Read the model definition and answer for the solid it produces. Units are mm, in the model's axes. Face numbers are marked on the shaded views. A direction names the side the tool comes from. Give positions to 0.01 mm unless a question says otherwise; leave off trailing zeros. Write each loop counter-clockwise with the first axis right and the second up, starting at its lowest first coordinate (ties: lowest second). Pieces come first, ordered by that corner, then holes. Notation, with made-up numbers: (33.25, -24.75) -> (74.25, -24.75) arc R22 ccw to (74.25, -16.75) -> close; hole circle Ø1 at (62, 11). An arc over 180 degrees is marked (long way). Answer as CSV lines item,"result". Start each with the question number.
1. Given pin 1 (1 mm diameter, centred on y = 10, z = -2, fed in from -X); pin 2 (1 mm diameter, centred on x = -2.5, y = 13.5, fed in from +Z); pin 3 (1 mm diameter, centred on y = 12.5, z = -2.5, fed in from +X), each flat-ended and moving along its own axis, determine where each tip first touches the part or whether it passes through.
2. The part is cut by section A-A, the plane y = 8.5. Determine the outline of the cut face in (x, z).
3. Find the intervals of material crossed by line 1 (Y direction, x = -3, z = -3.5); line 2 (X direction, y = 12.25, z = -2.5); line 3 (Z direction, x = -2, y = 5.5), in increasing order.
4. The part is cut by section B-B, the plane y = 12.5. Determine the outline of the cut face in (x, z).
5. The part is cut by section C-C, the plane y = 5. Determine the outline of the cut face in (x, z).
6. A tool of negligible diameter and unlimited length cuts with its end or side. For the marked faces 1, 2 and 3, from which of +Z, -Z, +X, -X, +Y, -Y can it reach the whole face along a straight path? Write none if from no direction.
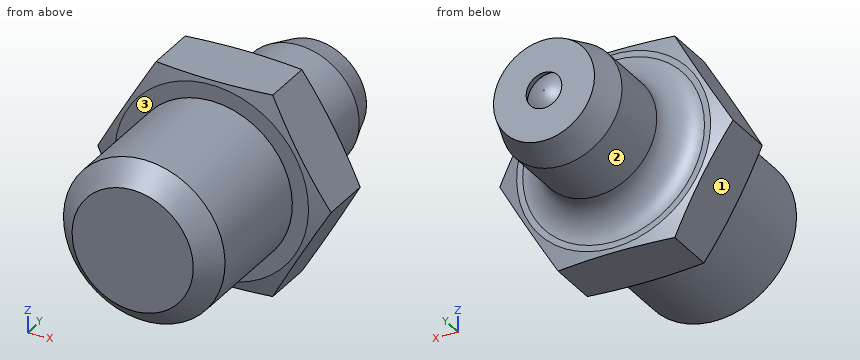
from build123d import *

# Parameters (mm, degrees)
SKETCH1_R           = 4
BOSS_EXTRUDE1_DEPTH = 6.8
BOSS_EXTRUDE2_DEPTH = 3
CHAMFER1_SIZE       = 1


with BuildPart() as part:
    # Sketch1 → Boss-Extrude1 (new body)
    with BuildSketch(Plane(origin=(0, 0, 0), x_dir=(1, 0, 0), z_dir=(0, 1, 0))):
        with Locations(Location((0, 0, 0), (0, 0, 270))):
            Circle(SKETCH1_R)
    extrude(amount=BOSS_EXTRUDE1_DEPTH)

    # Sketch2 → Boss-Extrude2 (add)
    with BuildSketch(Plane(origin=(0, 6.8, 0), x_dir=(1, 0, 0), z_dir=(0, 1, 0))):
        Polygon((2.886751346, -5), (5.773502692, 0), (2.886751346, 5), (-2.886751346, 5), (-5.773502692, 0), (-2.886751346, -5), align=None)
    extrude(amount=BOSS_EXTRUDE2_DEPTH)

    # Sketch3 → Revolve1 (revolve)
    with BuildSketch(Plane.XY, mode=Mode.PRIVATE) as revolve1_sk:
        with BuildLine():
            Line((0, 15.8), (0, 9.8))
            Line((0, 9.8), (4.500264384, 9.8))
            ThreePointArc((4.500264384, 9.8), (3.439434496, 10.239233666), (3, 11.29998038))
            Line((3, 11.29998038), (3, 14.3))
            Line((3, 14.3), (2.5, 15.8))
            Line((2.5, 15.8), (0, 15.8))
        make_face()
    revolve(revolve1_sk.sketch.rotate(Axis((0, -1.880404244, 0), (0, 1, 0)), 90), axis=Axis((0, -1.880404244, 0), (0, 1, 0)))

    # Sketch5 → Cut-Revolve1 (revolve, cut)
    with BuildSketch(Plane(origin=(0, 0, 0), x_dir=(0, 0, -1), z_dir=(1, 0, 0)), mode=Mode.PRIVATE) as cut_revolve1_sk:
        Polygon((-6.8, 9.8), (-4.8, 9.8), (-6.8, 9.3), align=None)
        Polygon((-6.8, 7.3), (-4.8, 6.8), (-6.8, 6.8), align=None)
    revolve(cut_revolve1_sk.sketch.rotate(Axis((0, 16.999618754, 0), (0, -1, 0)), 209.999999988), axis=Axis((0, 16.999618754, 0), (0, -1, 0)), mode=Mode.SUBTRACT)

    # Chamfer1
    chamfer1_edges = [part.edges().sort_by_distance(p)[0] for p in [
        (0, 0, -4),
    ]]
    chamfer(chamfer1_edges, length=CHAMFER1_SIZE)

    # Sketch6 → Cut-Revolve4 (revolve, cut)
    with BuildSketch(Plane(origin=(0, 0, 0), x_dir=(0, 0, -1), z_dir=(1, 0, 0))):
        with BuildLine():
            ThreePointArc((-1.292971656, 15.018429463), (-0.764043535, 15.584287943), (-0.02011539, 15.8))
            Line((-0.02011539, 15.8), (-0.882862678, 15.8))
            Line((-0.882862678, 15.8), (-1.292971656, 15.018429463))
        make_face()
    revolve(axis=Axis((0, 16.917153181, 0), (0, -1, 0)), mode=Mode.SUBTRACT)


solid = part.part
Results found:
1,pin 1,"stops at x = -4.86"
1,pin 2,"stops at z = 2.24"
1,pin 3,"stops at x = 2.24"
2,outline,"(-5.77, 0) -> (-2.89, -5) -> (2.89, -5) -> (5.77, 0) -> (2.89, 5) -> (-2.89, 5) -> close"
3,line 1,"y = 6.8 to 9.8"
3,line 2,"x = -1.66 to 1.66"
3,line 3,"z = -3.46 to 3.46"
4,outline,"circle Ø6 at (0, 0)"
5,outline,"circle Ø8 at (0, 0)"
6,face 1,"-Z, -X, +Y, -Y"
6,face 2,"+Y"
6,face 3,"-Y"
